Work out the finished part from the listing and answer in its coordinate system (mm). Face numbers are marked on the shaded views. Round coordinates to 2 decimals unless told otherwise and drop trailing zeros. Write each loop counter-clockwise with the first axis right and the second up, starting at its lowest first coordinate (ties: lowest second). Pieces come first, ordered by that corner, then holes.
1. Flat-ended cylindrical pins translate along their axes: pin 1 Ø2 at (x, z) = (2.5, -18) entering from -Y; pin 2 Ø10 at (x, y) = (5.5, -9) entering from -Z; pin 3 Ø5 at (x, z) = (1, -42.5) entering from +Y. Find the tip coordinate at first contact, or state that the pin passes through.
2. Determine the mould class of the marked faces 1, 2 and 3 for opening direction Z: pulls with the +Z half, pulls with the -Z half, needs draft (parallel to the pull), parting line crosses it, or undercut.
3. Find section A-A (x = 0). Write down the section's boundary in (y, z).
4. Find section C-C (y = -28). Write down the section's boundary in (x, z), and give its area (3 significant figures).
5. Find section B-B (z = -8). Write down the section's boundary in (x, y).
6. Straight lines are drawn through the part: probe 1 along Y at (x, z) = (0, -16.75); probe 2 along Z at (x, y) = (0.5, -28). For each, find the intervals that lie inside material, in ascending order.
```python
from build123d import *

# Parameters (mm, degrees)
SKETCH1_R          = 11
SKETCH1_R_2        = 9
CUT_EXTRUDE1_DEPTH = 25


with BuildPart() as part:
    # Sweep1: sweep along a path in Sketch2
    with BuildLine(Plane(origin=(0, 0, 0), x_dir=(0, 0, -1), z_dir=(1, 0, 0))) as sweep1_path:
        Line((0, 0), (30, 0))
        ThreePointArc((30, 0), (44.142135624, -5.857864376), (50, -20))
        Line((50, -20), (50, -150))
    # Sketch1 → Sweep1 (sweep)
    with BuildSketch(Plane.XY):
        Circle(SKETCH1_R)
        Circle(SKETCH1_R_2, mode=Mode.SUBTRACT)
    sweep(path=sweep1_path.line)

    # Sketch3 → Cut-Extrude1 (cut, symmetric)
    with BuildSketch(Plane(origin=(0, 0, 0), x_dir=(0, 0, -1), z_dir=(1, 0, 0))):
        Polygon((61, -150), (36.244444784, -125.244444784), (36.244444784, -150), align=None)
    extrude(amount=CUT_EXTRUDE1_DEPTH, both=True, mode=Mode.SUBTRACT)


solid = part.part
```
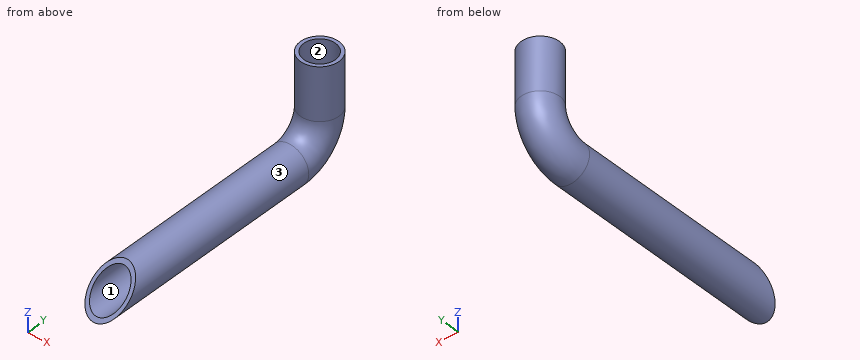
Worked answers:
1. pin 1: stops at y = -10.9
1. pin 2: stops at z = -59.91
1. pin 3: stops at y = 9.31
2. face 1: undercut
2. face 2: needs draft
2. face 3: parting line crosses it
3. outline: (-150, -61) - (-20, -61) arc R31 ccw to (11, -30) - (11, 0) - (9, 0) - (9, -30) arc R29 cw to (-20, -59) - (-148, -59) - close; (-130, -41) - (-20, -41) arc R11 ccw to (-9, -30) - (-9, 0) - (-11, 0) - (-11, -30) arc R9 cw to (-20, -39) - (-128, -39) - close
4. outline: circle Ø22 at (0, -50); hole circle Ø18 at (0, -50)
4. area: 126 mm2
5. outline: circle Ø22 at (0, 0); hole circle Ø18 at (0, 0)
6. probe 1: y = -11 to -9, 9 to 11
6. probe 2: z = -60.99 to -58.99, -41.01 to -39.01
